The listing builds one solid part. Answer for the finished solid, in the listing's coordinates (mm). Round coordinates to 2 decimals unless told otherwise and drop trailing zeros. Order: outer loops, then holes, each group sorted by start corner. A loop starts at its lowest first (then second) coordinate and runs counter-clockwise, first axis right, second up. Notation, with made-up numbers: (53.5, -18.75) - (65.5, -18.75) arc R19 cw to (65.5, -4.75) - close; hole circle Ø2 at (59, 66). An arc over 180 degrees is marked (long way). Write item = value, one per line.
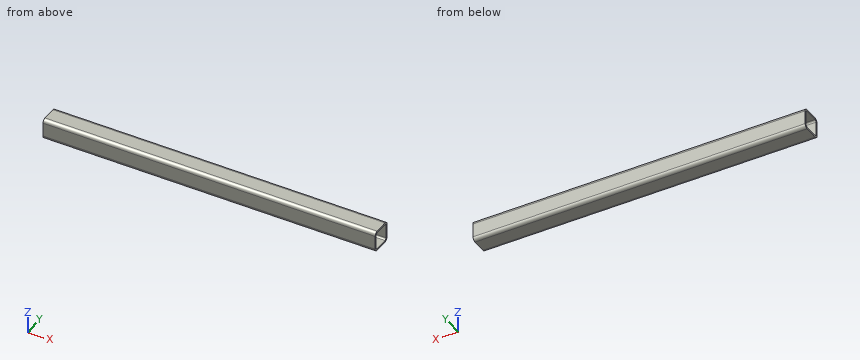
from build123d import *

# Parameters (mm, degrees)
SQUARE_TUBE_30_X_30_X_2_5_DEPTH = 480


with BuildPart() as part:
    # Sketch16 → Square tube 30 X 30 X 2.5 (new body)
    with BuildSketch(Plane.YZ.offset(-240)):
        with BuildLine():
            Line((-10, -15), (10, -15))
            ThreePointArc((10, -15), (13.535533906, -13.535533906), (15, -10))
            Line((15, -10), (15, 10))
            ThreePointArc((15, 10), (13.535533906, 13.535533906), (10, 15))
            Line((10, 15), (-10, 15))
            ThreePointArc((-10, 15), (-13.535533906, 13.535533906), (-15, 10))
            Line((-15, 10), (-15, -10))
            ThreePointArc((-15, -10), (-13.535533906, -13.535533906), (-10, -15))
        make_face()
        with BuildLine():
            Line((-10, -12.5), (10, -12.5))
            ThreePointArc((10, -12.5), (11.767766953, -11.767766953), (12.5, -10))
            Line((12.5, -10), (12.5, 10))
            ThreePointArc((12.5, 10), (11.767766953, 11.767766953), (10, 12.5))
            Line((10, 12.5), (-10, 12.5))
            ThreePointArc((-10, 12.5), (-11.767766953, 11.767766953), (-12.5, 10))
            Line((-12.5, 10), (-12.5, -10))
            ThreePointArc((-12.5, -10), (-11.767766953, -11.767766953), (-10, -12.5))
        make_face(mode=Mode.SUBTRACT)
    extrude(amount=SQUARE_TUBE_30_X_30_X_2_5_DEPTH)


solid = part.part
Q1. A flat-ended cylindrical pin translates along its axis: P1, Ø6, axis at y = 9, z = -0.5, coming from the -X side. Find the tip coordinate at first contact, or state that the pin passes through.
Model answer:
P1 = through
Q2. Section A-A on y = 5 is taken. Determine the outline of the cut face in (x, z), then the cut area to 3 significant figures.
Model answer:
outline = (-240, -15) - (240, -15) - (240, -12.5) - (-240, -12.5) - close; (-240, 12.5) - (240, 12.5) - (240, 15) - (-240, 15) - close
area = 2,400 mm^2
Q3. Section B-B on x = -93 is taken. Determine the outline of the cut face in (y, z), then the cut area to 3 significant figures.
Model answer:
outline = (-15, -10) arc R5 ccw to (-10, -15) - (10, -15) arc R5 ccw to (15, -10) - (15, 10) arc R5 ccw to (10, 15) - (-10, 15) arc R5 ccw to (-15, 10) - close; hole (-12.5, -10) arc R2.5 ccw to (-10, -12.5) - (10, -12.5) arc R2.5 ccw to (12.5, -10) - (12.5, 10) arc R2.5 ccw to (10, 12.5) - (-10, 12.5) arc R2.5 ccw to (-12.5, 10) - close
area = 259 mm^2
Q4. Find the intervals of material crossed by line 1 (Y direction, x = 144, z = -3.75); line 2 (Z direction, x = -102.5, y = 11.75), in increasing order. Write a range as from..to.
Model answer:
line_1 = -15..-12.5, 12.5..15
line_2 = -14.68..-11.79, 11.79..14.68
